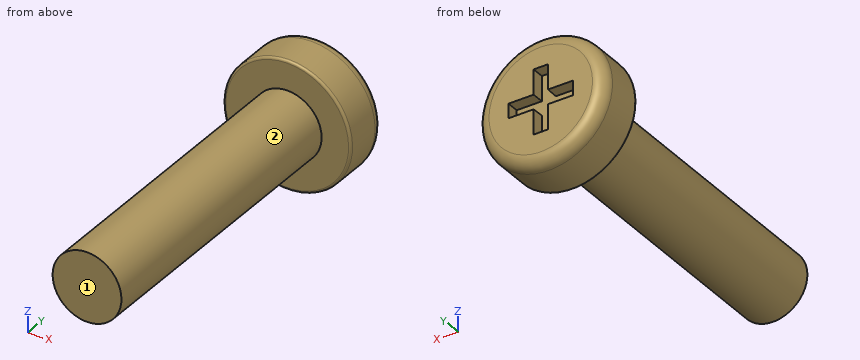
from build123d import *

# Parameters (mm, degrees)
SKETCH1_R           = 2.65
BOSS_EXTRUDE1_DEPTH = 2
SKETCH2_R           = 1.43
BOSS_EXTRUDE2_DEPTH = 12.5
FILLET1_R           = 0.5
FILLET2_R           = 0.1
CUT_EXTRUDE1_DEPTH  = 0.5
CUT_EXTRUDE1_DRAFT  = -1


with BuildPart() as part:
    # Sketch1 → Boss-Extrude1 (new body)
    with BuildSketch(Plane(origin=(0, 0, 0), x_dir=(1, 0, 0), z_dir=(0, 1, 0))):
        with Locations(Location((0, 0, 0), (0, 0, 270))):
            Circle(SKETCH1_R)
    extrude(amount=BOSS_EXTRUDE1_DEPTH)

    # Sketch2 → Boss-Extrude2 (add)
    with BuildSketch(Plane.XZ):
        with Locations(Location((0, 0, 0), (0, 0, 90))):
            Circle(SKETCH2_R)
    extrude(amount=BOSS_EXTRUDE2_DEPTH)

    # Fillet1
    fillet1_edges = [part.edges().sort_by_distance(p)[0] for p in [
        (0, 2, -2.65),
    ]]
    fillet(fillet1_edges, radius=FILLET1_R)

    # Fillet2
    fillet2_edges = [part.edges().sort_by_distance(p)[0] for p in [
        (0, 0, -2.65),
    ]]
    fillet(fillet2_edges, radius=FILLET2_R)


with BuildPart() as cut_extrude1_tool:
    # Sketch3 → Cut-Extrude1 (with draft: the straight prism first)
    with BuildSketch(Plane(origin=(0, 2, 0), x_dir=(1, 0, 0), z_dir=(0, 1, 0))):
        Polygon((0.296573117, 0.3), (0.296573117, 1.336133674), (-0.303426883, 1.336133674), (-0.303426883, 0.3), (-1.340662941, 0.3), (-1.340662941, -0.3), (-0.303426883, -0.3), (-0.303426883, -1.336133674), (0.296573117, -1.336133674), (0.296573117, -0.3), (1.340662941, -0.3), (1.340662941, 0.3), align=None)
    extrude(amount=-CUT_EXTRUDE1_DEPTH)
    # Cut-Extrude1: the draft: its side faces are tilted about the plane it starts from
    cut_extrude1_sides = [cut_extrude1_tool.faces().sort_by_distance(p)[0] for p in [
        (0.296573117, 1.75, -0.818066837),
        (-0.003426883, 1.75, -1.336133674),
        (-0.303426883, 1.75, -0.818066837),
        (-0.822044912, 1.75, -0.3),
        (-1.340662941, 1.75, 0),
        (-0.822044912, 1.75, 0.3),
        (-0.303426883, 1.75, 0.818066837),
        (-0.003426883, 1.75, 1.336133674),
        (0.296573117, 1.75, 0.818066837),
        (0.818618029, 1.75, 0.3),
        (1.340662941, 1.75, 0),
        (0.818618029, 1.75, -0.3),
    ]]
    draft(cut_extrude1_sides, Plane(origin=(0, 2, 0), x_dir=(1, 0, 0), z_dir=(0, 1, 0)), CUT_EXTRUDE1_DRAFT)


with BuildPart() as part_1:
    add(part.part)

    # Cut-Extrude1: cut by cut_extrude1_tool
    add(cut_extrude1_tool.part, mode=Mode.SUBTRACT)


solid = part_1.part
CAD build for the part. Positions are in the model's coordinates, mm. Face numbers are marked on the shaded views. A direction names the side the tool comes from. Coordinates: 2 decimals unless noted, no trailing zeros. Order: outer loops, then holes, each group sorted by start corner. A loop starts at its lowest first (then second) coordinate and runs counter-clockwise, first axis right, second up.
Item 1: Band-saw the part on A-A on x = 0. List the corners of the cut face in (y, z).
Check sheet entries:
outline: (-12.5, -1.43) - (0, -1.43) - (0, -2.55) arc R0.1 ccw to (0.1, -2.65) - (1.5, -2.65) arc R0.5 ccw to (2, -2.15) - (2, -1.34) - (1.5, -1.33) - (1.5, 1.33) - (2, 1.34) - (2, 2.15) arc R0.5 ccw to (1.5, 2.65) - (0.1, 2.65) arc R0.1 ccw to (0, 2.55) - (0, 1.43) - (-12.5, 1.43) - close
Item 2: Drill centre lines: L1, parallel to Y at x = 0.85, z = -1.2; L2, parallel to Z at x = 0.5, y = -10; L3, parallel to Y at x = -0.4, z = -2.35. Where is each one in solid material? Low to high.
Check sheet entries:
L1: y = 0 to 2
L2: z = -1.34 to 1.34
L3: y = 0 to 1.94
Item 3: Band-saw the part on B-B on z = 0. List the corners of the cut face in (x, y), plus the area to 3 significant figures.
Check sheet entries:
outline: (-2.65, 0.1) arc R0.1 ccw to (-2.55, 0) - (-1.43, 0) - (-1.43, -12.5) - (1.43, -12.5) - (1.43, 0) - (2.55, 0) arc R0.1 ccw to (2.65, 0.1) - (2.65, 1.5) arc R0.5 ccw to (2.15, 2) - (1.34, 2) - (1.33, 1.5) - (-1.33, 1.5) - (-1.34, 2) - (-2.15, 2) arc R0.5 ccw to (-2.65, 1.5) - close
area: 44.9 mm2
Item 4: 3-axis set-ups, long thin cutter, end or side, ignore diameter. For the marked faces 1 and 2: which of +Z, -Z, +X, -X, +Y, -Y reach the whole face in a straight line?
Check sheet entries:
face 1: +Z, -Z, +X, -X, -Y
face 2: -Y
Item 5: Band-saw the part on C-C on y = -5.75. List the corners of the cut face in (x, z), plus the area to 3 significant figures.
Check sheet entries:
outline: circle Ø2.86 at (0, 0)
area: 6.42 mm2
Item 6: Pin check, flat tips, straight feed: pin 1 Ø1.5 at (x, y) = (-0.5, -4) entering from -Z; pin 2 Ø2 at (x, z) = (-2, -1) entering from +Y; pin 3 Ø1 at (x, y) = (-1.5, 0) entering from -Z; pin 4 Ø1 at (y, z) = (-2.5, 0) entering from +X. Stop position of each tip, or through.
Check sheet entries:
pin 1: stops at z = -1.43
pin 2: stops at y = 2
pin 3: stops at z = -2.45
pin 4: stops at x = 1.43
Item 7: Band-saw the part on D-D on y = 0.25. List the corners of the cut face in (x, z).
Check sheet entries:
outline: circle Ø5.3 at (0, 0)
